Input: part model. Units: mm. Frame: model coordinates. A direction names the side the tool comes from. Round coordinates to 2 decimals unless told otherwise and drop trailing zeros. Order: outer loops, then holes, each group sorted by start corner. A loop starts at its lowest first (then second) coordinate and runs counter-clockwise, first axis right, second up.
Item 1: Cut plane C-C on x = -10.5. Output: boundary loops of the cut face in (y, z), then the cut area to 3 significant figures.
Item 2: Line query: L1, parallel to Y at x = -17, z = 12.25; L2, parallel to Y at x = 0, z = 13.6; L3, parallel to X at y = 6, z = 14.25. Output: solid intervals per line, ascending.
Item 3: First-contact query: pin 1 (2 mm diameter, centred on y = 6, z = 2, fed in from -X); pin 2 (5 mm diameter, centred on x = -17.5, y = 2.5, fed in from -Z); pin 3 (4 mm diameter, centred on x = 0, y = 0, fed in from +Z); pin 4 (1.6 mm diameter, centred on x = 0, y = 0, fed in from +Z). Flat tips, straight axial feed; report the tip coordinate or a pass-through.
Item 4: Cut plane B-B on z = 9.25. Output: boundary loops of the cut face in (x, y).
Item 5: Cut plane D-D on z = 14.5. Output: boundary loops of the cut face in (x, y).
Item 6: Mould query, pull axis X, two halves, no side actions, for faces 6 (the flat face through (-10, -10, 12)), 7 (the flat face through (-25, 0, 12)), 8 (the cylindrical face through (-6.9, 6, 12.6)). Classes: released by +X, released by -X, zero draft, split by the parting line, or undercut.
Item 7: Cut plane A-A on y = 6. Output: boundary loops of the cut face in (x, z).
Item 8: Reachability of faces 1 (the flat face through (-5, 0, 4)), 2 (the cylindrical face through (4.715, -3.699, 4.056)), 3 (the flat face through (0, 4, 4)), 4 (the flat face through (-15, -8.1, 13)), 5 (the flat face through (0, -4, 4)) from +Z, -Z, +X, -X, +Y, -Y: full face, straight path, thin tool, end or side. Return the list, or none.
```python
from build123d import *

# Parameters (mm, degrees)
SKETCH_1_W          = 10
SKETCH_1_H          = 8
EXTRUDE_1_DEPTH     = 8
SKETCH_2_W          = 10
SKETCH_2_H          = 20
EXTRUDE_2_DEPTH     = 9
SKETCH_4_R          = 1.65
CUT_EXTRUDE_2_DEPTH = 6
SKETCH_7_W          = 9
SKETCH_7_H          = 20
EXTRUDE_3_DEPTH     = 20
CUT_EXTRUDE_5_DEPTH = 20
FILLET_2_R          = 2
FILLET_3_R          = 1


with BuildPart() as part:
    # 草图1 → 凸台-拉伸1 (new body)
    with BuildSketch(Plane.XY):
        Rectangle(SKETCH_1_W, SKETCH_1_H)
    extrude(amount=EXTRUDE_1_DEPTH)

    # 草图2 → 凸台-拉伸2 (add)
    with BuildSketch(Plane.XY.offset(8)):
        Rectangle(SKETCH_2_W, SKETCH_2_H)
    extrude(amount=EXTRUDE_2_DEPTH)

    # 草图4 → 切除-拉伸2 (cut)
    with BuildSketch(Plane.XY.offset(17)):
        Circle(SKETCH_4_R)
    extrude(amount=-CUT_EXTRUDE_2_DEPTH, mode=Mode.SUBTRACT)

    # 草图7 → 凸台-拉伸3 (add)
    with BuildSketch(Plane.ZY.offset(5)):
        with Locations((12.5, 0)):
            Rectangle(SKETCH_7_W, SKETCH_7_H)
    extrude(amount=EXTRUDE_3_DEPTH)

    # 草图8 → 切除-拉伸5 (cut)
    with BuildSketch(Plane.XY.offset(17)):
        with BuildLine():
            Line((-21, 8.1), (-9, 8.1))
            ThreePointArc((-9, 8.1), (-6.9, 6), (-9, 3.9))
            Line((-9, 3.9), (-21, 3.9))
            ThreePointArc((-21, 3.9), (-23.1, 6), (-21, 8.1))
        make_face()
        with BuildLine():
            Line((-21, -8.1), (-9, -8.1))
            ThreePointArc((-9, -8.1), (-6.9, -6), (-9, -3.9))
            Line((-9, -3.9), (-21, -3.9))
            ThreePointArc((-21, -3.9), (-23.1, -6), (-21, -8.1))
        make_face()
    extrude(amount=-CUT_EXTRUDE_5_DEPTH, mode=Mode.SUBTRACT)

    # 圆角2
    fillet_2_edges = [part.edges().sort_by_distance(p)[0] for p in [
        (5, -10, 12.5),
        (5, 10, 12.5),
        (-25, -10, 12.5),
        (-25, 10, 12.5),
    ]]
    fillet(fillet_2_edges, radius=FILLET_2_R)

    # 圆角3
    fillet_3_edges = [part.edges().sort_by_distance(p)[0] for p in [
        (5, -4, 4),
        (-5, -4, 4),
        (-5, 4, 4),
        (5, 4, 4),
    ]]
    fillet(fillet_3_edges, radius=FILLET_3_R)


solid = part.part
```
From the geometry:
1. outline: (-10, 8) - (-8.1, 8) - (-8.1, 17) - (-10, 17) - close; (-3.9, 8) - (3.9, 8) - (3.9, 17) - (-3.9, 17) - close; (8.1, 8) - (10, 8) - (10, 17) - (8.1, 17) - close
1. area: 104 mm2
2. L1: y = -10 to -8.1, -3.9 to 3.9, 8.1 to 10
2. L2: y = -10 to -1.65, 1.65 to 10
2. L3: x = -25 to -23.1, -6.9 to 5
3. pin 1: passes through
3. pin 2: stops at z = 8
3. pin 3: stops at z = 17
3. pin 4: stops at z = 11
4. outline: (-25, -8) arc R2 ccw to (-23, -10) - (3, -10) arc R2 ccw to (5, -8) - (5, 8) arc R2 ccw to (3, 10) - (-23, 10) arc R2 ccw to (-25, 8) - close; hole (-21, -8.1) - (-9, -8.1) arc R2.1 ccw to (-9, -3.9) - (-21, -3.9) arc R2.1 ccw to start; hole (-21, 3.9) - (-9, 3.9) arc R2.1 ccw to (-9, 8.1) - (-21, 8.1) arc R2.1 ccw to start
5. outline: (-25, -8) arc R2 ccw to (-23, -10) - (3, -10) arc R2 ccw to (5, -8) - (5, 8) arc R2 ccw to (3, 10) - (-23, 10) arc R2 ccw to (-25, 8) - close; hole (-21, -8.1) - (-9, -8.1) arc R2.1 ccw to (-9, -3.9) - (-21, -3.9) arc R2.1 ccw to start; hole (-21, 3.9) - (-9, 3.9) arc R2.1 ccw to (-9, 8.1) - (-21, 8.1) arc R2.1 ccw to start; hole circle Ø3.3 at (0, 0)
6. face 6: zero draft
6. face 7: released by -X
6. face 8: undercut
7. outline: (-25, 8) - (-23.1, 8) - (-23.1, 17) - (-25, 17) - close; (-6.9, 8) - (5, 8) - (5, 17) - (-6.9, 17) - close
8. face 1: -Z, -X, +Y, -Y
8. face 2: -Z, +X, -Y
8. face 3: -Z, +X, -X, +Y
8. face 4: +Z, -Z
8. face 5: -Z, +X, -X, -Y
